The listing builds one solid part. Answer for the finished solid, in the listing's coordinates (mm). Face numbers are marked on the shaded views. Give positions to 0.01 mm unless a question says otherwise; leave off trailing zeros. Order: outer loops, then holes, each group sorted by start corner. A loop starts at its lowest first (then second) coordinate and runs counter-clockwise, first axis right, second up. Notation, with made-up numbers: (81, 13.5) - (106, 13.5) arc R26 ccw to (106, 42.5) - close; hole circle Ø9 at (53, -10.75). An arc over 180 degrees is marked (long way). Answer as a JSON object with one key per item and string values. Group by question number.
Q1. A cutting plane is placed at D-D, the plane y = 5.5. Give the vertices of the cut face in (x, z), and give its area (3 significant figures).
Q2. A cutting plane is placed at A-A, the plane z = 20. Give the vertices of the cut face in (x, y).
Q3. A cutting plane is placed at B-B, the plane y = 19.25. Give the vertices of the cut face in (x, z), and give its area (3 significant figures).
Q4. A cutting plane is placed at C-C, the plane x = 42.5. Give the vertices of the cut face in (y, z), and give its area (3 significant figures).
Q5. Consider line 1 (Z direction, x = 64, y = 1.5); line 2 (X direction, y = 21.5, z = 19.5); line 3 (Y direction, x = 86, z = 79.5). Determine where each line is inside the solid, lowest interval first.
Q6. Given pin 1 (1 mm diameter, centred on x = 13.5, z = 23.5, fed in from +Y), flat-ended and moving along its own axis, determine where the tip first touches the part or whether it passes through.
Q7. The mould has two halves that part along X. Classify the marked faces 1, 2, 3 and 4: released by +X, released by -X, zero draft, split by the parting line, or undercut.
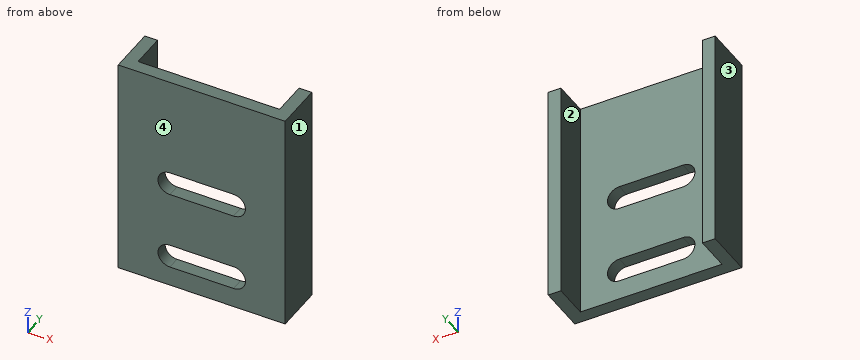
from build123d import *

# Parameters (mm, degrees)
EXTRUDE_1_DEPTH     = 140
CUT_EXTRUDE_1_DEPTH = 140


with BuildPart() as part:
    # 草图1 → 凸台-拉伸1 (new body)
    with BuildSketch(Plane.XY):
        Polygon((0, 0), (105, 0), (105, 30), (97, 30), (97, 8), (8, 8), (8, 30), (0, 30), align=None)
    extrude(amount=EXTRUDE_1_DEPTH)

    # 草图2 → 切除-拉伸1 (cut)
    with BuildSketch(Plane.XZ):
        with BuildLine():
            Line((52.5, 70), (52.5, 62.5))
            Line((52.5, 62.5), (72.5, 62.5))
            ThreePointArc((72.5, 62.5), (80, 70), (72.5, 77.5))
            Line((72.5, 77.5), (52.5, 77.5))
            Line((52.5, 77.5), (52.5, 70))
        make_face()
        with BuildLine():
            Line((32.5, 62.5), (52.5, 62.5))
            Line((52.5, 62.5), (52.5, 70))
            Line((52.5, 70), (52.5, 77.5))
            Line((52.5, 77.5), (32.5, 77.5))
            ThreePointArc((32.5, 77.5), (25, 70), (32.5, 62.5))
        make_face()
        with BuildLine():
            Line((32.5, 12.5), (52.5, 12.5))
            Line((52.5, 12.5), (52.5, 20))
            Line((52.5, 20), (52.5, 27.5))
            Line((52.5, 27.5), (32.5, 27.5))
            ThreePointArc((32.5, 27.5), (25, 20), (32.5, 12.5))
        make_face()
        with BuildLine():
            Line((52.5, 20), (52.5, 12.5))
            Line((52.5, 12.5), (72.5, 12.5))
            ThreePointArc((72.5, 12.5), (80, 20), (72.5, 27.5))
            Line((72.5, 27.5), (52.5, 27.5))
            Line((52.5, 27.5), (52.5, 20))
        make_face()
    extrude(amount=-CUT_EXTRUDE_1_DEPTH, mode=Mode.SUBTRACT)


solid = part.part
Reply:
{
 "1": {"outline": "(0, 0) - (105, 0) - (105, 140) - (0, 140) - close; hole (32.5, 12.5) - (72.5, 12.5) arc R7.5 ccw to (72.5, 27.5) - (32.5, 27.5) arc R7.5 ccw to start; hole (32.5, 62.5) - (72.5, 62.5) arc R7.5 ccw to (72.5, 77.5) - (32.5, 77.5) arc R7.5 ccw to start", "area": "13,100 mm^2"},
 "2": {"outline": "(0, 0) - (25, 0) - (25, 8) - (8, 8) - (8, 30) - (0, 30) - close; (80, 0) - (105, 0) - (105, 30) - (97, 30) - (97, 8) - (80, 8) - close"},
 "3": {"outline": "(0, 0) - (8, 0) - (8, 140) - (0, 140) - close; (97, 0) - (105, 0) - (105, 140) - (97, 140) - close", "area": "2,240 mm^2"},
 "4": {"outline": "(0, 0) - (8, 0) - (8, 12.5) - (0, 12.5) - close; (0, 27.5) - (8, 27.5) - (8, 62.5) - (0, 62.5) - close; (0, 77.5) - (8, 77.5) - (8, 140) - (0, 140) - close", "area": "880 mm^2"},
 "5": {"line 1": "z = 0 to 12.5, 27.5 to 62.5, 77.5 to 140", "line 2": "x = 0 to 8, 97 to 105", "line 3": "y = 0 to 8"},
 "6": {"pin 1": "stops at y = 8"},
 "7": {"face 1": "released by +X", "face 2": "undercut", "face 3": "released by -X", "face 4": "zero draft"}
}
